```python
from build123d import *

# Parameters (mm, degrees)
EXTRUDE_1182_DEPTH                  = 20
SKETCH_1261_R                       = 9.7
SKETCH_1261_R_2                     = 8
EXTRUDE_1314_DEPTH                  = 25
EXTRUDE_1314_DIRECTION_2_REACH      = 36.873
EXTRUDE_1314_DIRECTION_2_END_RADIUS = 57.25
CUT_EXTRUDE_1_DEPTH                 = 54.783006673
CUT_EXTRUDE_1_DEPTH_BACK            = 54.783006673


with BuildPart() as part:
    # Sketch 176 → Extrude 1182 (new, symmetric)
    with BuildSketch(Plane.XY):
        with BuildLine():
            ThreePointArc((-7.173913043, 24.16738193), (-14.079724741, 13.582112358), (-16.5, 1.177257067))
            ThreePointArc((-16.5, 1.177257067), (0, -1.2), (16.5, 1.177257067))
            ThreePointArc((16.5, 1.177257067), (14.079724741, 13.582112358), (7.173913043, 24.16738193))
            ThreePointArc((7.173913043, 24.16738193), (0, 27.200677426), (-7.173913043, 24.16738193))
        make_face()
        with BuildLine():
            ThreePointArc((-0.89349881, 14.363604773), (-3.663033007, 7.517669831), (-4.022846329, 0.141513701))
            ThreePointArc((-4.022846329, 0.141513701), (-9.556707772, 0.803283208), (-15, 2))
            ThreePointArc((-15, 2), (-13.262165522, 12.062305899), (-8.25, 20.95883699))
            ThreePointArc((-8.25, 20.95883699), (-4.170568058, 18.108709455), (-0.89349881, 14.363604773))
        make_face(mode=Mode.SUBTRACT)
        with BuildLine():
            ThreePointArc((-2.5, 0.0546112), (-2.301572456, 6.695550977), (0, 12.928064021))
            ThreePointArc((0, 12.928064021), (2.301572456, 6.695550977), (2.5, 0.0546112))
            ThreePointArc((2.5, 0.0546112), (0, 0), (-2.5, 0.0546112))
        make_face(mode=Mode.SUBTRACT)
        with BuildLine():
            ThreePointArc((4.022846329, 0.141513701), (3.663033007, 7.517669831), (0.89349881, 14.363604773))
            ThreePointArc((0.89349881, 14.363604773), (4.170568058, 18.108709455), (8.25, 20.95883699))
            ThreePointArc((8.25, 20.95883699), (13.262165522, 12.062305899), (15, 2))
            ThreePointArc((15, 2), (9.556707772, 0.803283208), (4.022846329, 0.141513701))
        make_face(mode=Mode.SUBTRACT)
        with BuildLine():
            ThreePointArc((7.245751005, 22.120715085), (3.267177029, 19.312833939), (0, 15.701905849))
            ThreePointArc((0, 15.701905849), (-3.267177029, 19.312833939), (-7.245751005, 22.120715085))
            ThreePointArc((-7.245751005, 22.120715085), (0, 25.228756555), (7.245751005, 22.120715085))
        make_face(mode=Mode.SUBTRACT)
    extrude(amount=EXTRUDE_1182_DEPTH, both=True)

    # Sketch 1261 → Extrude 1314 (add)
    with BuildSketch(Plane(origin=(0, 22.120715085, 0), x_dir=(-1, 0, 0), z_dir=(0, -1, 0))):
        with Locations(Location((0, 0, 0), (0, 0, 222.304463408))):
            Circle(SKETCH_1261_R)
        with Locations(Location((0, 0, 0), (0, 0, 206.267303198))):
            Circle(SKETCH_1261_R_2, mode=Mode.SUBTRACT)
    extrude(amount=-EXTRUDE_1314_DEPTH)

    # Extrude 1314 direction 2: up to this cylinder (the profile starts inside it)
    extrude_1314_direction_2_end = Plane(origin=(0, 57.25, -6.344118), z_dir=(0, 0, -1)) * Cylinder(EXTRUDE_1314_DIRECTION_2_END_RADIUS, 189.246, mode=Mode.PRIVATE)
    # Sketch 1261 → Extrude 1314 direction 2 (add, up to the surface)
    with BuildSketch(Plane(origin=(0, 22.120715085, 0), x_dir=(-1, 0, 0), z_dir=(0, -1, 0)), mode=Mode.PRIVATE) as extrude_1314_direction_2_sk1:
        with Locations(Location((0, 0, 0), (0, 0, 222.304463408))):
            Circle(SKETCH_1261_R)
        with Locations(Location((0, 0, 0), (0, 0, 206.267303198))):
            Circle(SKETCH_1261_R_2, mode=Mode.SUBTRACT)
    extrude_1314_direction_2_tool1 = extrude(extrude_1314_direction_2_sk1.sketch, amount=EXTRUDE_1314_DIRECTION_2_REACH, mode=Mode.PRIVATE) & extrude_1314_direction_2_end
    add(extrude_1314_direction_2_tool1.solids().sort_by_distance((-6.971004, 22.120715, -6.344118))[0])

    # Sketch 1375 → 切除-拉伸1 (cut, two sides: drawn at the far end of the back side and taken through both)
    with BuildSketch(Plane.XY.offset(-CUT_EXTRUDE_1_DEPTH_BACK)):
        with BuildLine():
            ThreePointArc((4.022846329, 0.141513701), (9.556707772, 0.803283208), (15, 2))
            ThreePointArc((15, 2), (13.262165522, 12.062305899), (8.25, 20.95883699))
            ThreePointArc((8.25, 20.95883699), (4.170568058, 18.108709455), (0.89349881, 14.363604773))
            ThreePointArc((0.89349881, 14.363604773), (3.663033007, 7.517669831), (4.022846329, 0.141513701))
        make_face()
        with BuildLine():
            ThreePointArc((-8.25, 20.95883699), (-13.262165522, 12.062305899), (-15, 2))
            ThreePointArc((-15, 2), (-9.556707772, 0.803283208), (-4.022846329, 0.141513701))
            ThreePointArc((-4.022846329, 0.141513701), (-3.663033007, 7.517669831), (-0.89349881, 14.363604773))
            ThreePointArc((-0.89349881, 14.363604773), (-4.170568058, 18.108709455), (-8.25, 20.95883699))
        make_face()
        with BuildLine():
            ThreePointArc((-2.5, 0.0546112), (0, 0), (2.5, 0.0546112))
            ThreePointArc((2.5, 0.0546112), (2.301572456, 6.695550977), (0, 12.928064021))
            ThreePointArc((0, 12.928064021), (-2.301572456, 6.695550977), (-2.5, 0.0546112))
        make_face()
        with BuildLine():
            ThreePointArc((7.245751005, 22.120715085), (3.267177029, 19.312833939), (0, 15.701905849))
            ThreePointArc((0, 15.701905849), (-3.267177029, 19.312833939), (-7.245751005, 22.120715085))
            ThreePointArc((-7.245751005, 22.120715085), (0, 25.228756555), (7.245751005, 22.120715085))
        make_face()
    extrude(amount=CUT_EXTRUDE_1_DEPTH + CUT_EXTRUDE_1_DEPTH_BACK, mode=Mode.SUBTRACT)


solid = part.part
```
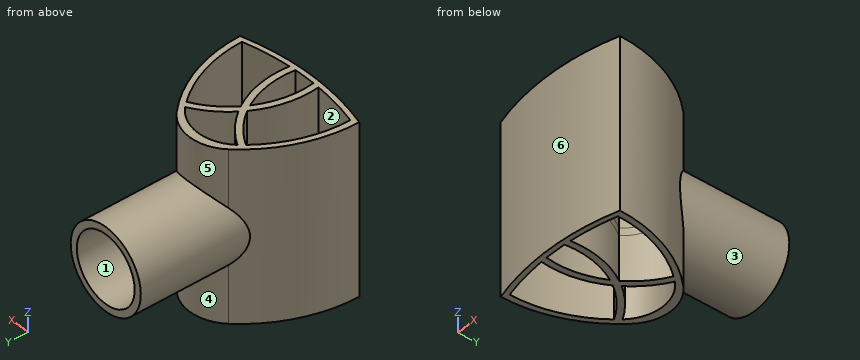
The listing builds one solid part. Answer for the finished solid, in the listing's coordinates (mm). Face numbers are marked on the shaded views. A direction names the side the tool comes from. Give positions to 0.01 mm unless a question says otherwise; leave off trailing zeros. Order: outer loops, then holes, each group sorted by start corner. A loop starts at its lowest first (then second) coordinate and runs counter-clockwise, first axis right, second up. Notation, with made-up numbers: (-27.5, 55) -> (-7.5, 55) arc R22 cw to (-7.5, 88) -> close; hole circle Ø3 at (76, 69.5). An arc over 180 degrees is marked (long way). One line per item, written item: value.
1) Flat-ended cylindrical pins translate along their axes: P1, Ø12, axis at x = 9.5, z = 1, coming from the -Y side; P2, Ø8, axis at x = 12, y = 34.5, coming from the -Z side; P3, Ø2, axis at x = -13, y = 11, coming from the +Z side; P4, Ø8, axis at y = 39, z = 2, coming from the +X side. Find the tip coordinate at first contact, or state that the pin passes through.
Reported:
P1: stops at y = -1.1
P2: stops at z = -5.49
P3: stops at z = 20
P4: stops at x = 9.7
2) Find section B-B, the plane y = 7.5. Determine the outline of the cut face in (x, z).
Reported:
outline: (-15.89, -20) -> (-14.49, -20) -> (-14.49, 20) -> (-15.89, 20) -> close; (-3.67, -20) -> (-2.13, -20) -> (-2.13, 20) -> (-3.67, 20) -> close; (2.13, -20) -> (3.67, -20) -> (3.67, 20) -> (2.13, 20) -> close; (14.49, -20) -> (15.89, -20) -> (15.89, 20) -> (14.49, 20) -> close
3) Find section A-A, the plane z = -13.5. Determine the outline of the cut face in (x, y).
Reported:
outline: (-16.5, 1.18) arc R58.45 ccw to (16.5, 1.18) arc R33 ccw to (7.17, 24.17) arc R10 ccw to (-7.17, 24.17) arc R33 ccw to start; hole (-15, 2) arc R57.25 ccw to (-4.02, 0.14) arc R22.1 cw to (-0.89, 14.36) arc R20.6 ccw to (-8.25, 20.96) arc R30 ccw to start; hole (-7.25, 22.12) arc R22.1 cw to (0, 15.7) arc R22.1 cw to (7.25, 22.12) arc R10 ccw to start; hole (-2.5, 0.05) arc R57.25 ccw to (2.5, 0.05) arc R20.6 ccw to (0, 12.93) arc R20.6 ccw to start; hole (0.89, 14.36) arc R22.1 cw to (4.02, 0.14) arc R57.25 ccw to (15, 2) arc R30 ccw to (8.25, 20.96) arc R20.6 ccw to start
4) Find section C-C, the plane x = -14. Determine the outline of the cut face in (y, z).
Reported:
outline: (0.5, -20) -> (1.74, -20) -> (1.74, 20) -> (0.5, 20) -> close; (9.68, -20) -> (13.78, -20) -> (13.78, 20) -> (9.68, 20) -> close
5) Determine the mould class of the marked faces 1, 2 and 3 for opening direction Z: pulls with the +Z half, pulls with the -Z half, needs draft (parallel to the pull), parting line crosses it, or undercut.
Reported:
face 1: undercut
face 2: needs draft
face 3: parting line crosses it
6) A tool of negligible diameter and unlimited length cuts with its end or side. For the marked faces 4, 5 and 6, from which of +Z, -Z, +X, -X, +Y, -Y can it reach the whole face along a straight path? Write none if from no direction.
Reported:
face 4: -Z, +Y
face 5: +Z, +Y
face 6: +Z, -Z, -Y
7) Find section D-D, the plane y = 13.5. Determine the outline of the cut face in (x, z), plus the area to 3 significant figures.
Reported:
outline: (-14.11, -20) -> (-12.71, -20) -> (-12.71, 20) -> (-14.11, 20) -> close; (-1.4, -20) -> (1.4, -20) -> (1.4, 20) -> (-1.4, 20) -> close; (12.71, -20) -> (14.11, -20) -> (14.11, 20) -> (12.71, 20) -> close
area: 224 mm^2
8) Find the intervals of material crossed by line 1 (X direction, y = 29, z = 0); line 2 (X direction, y = 7.5, z = -2.5), in increasing order.
Reported:
line 1: x = -9.7 to -8, 8 to 9.7
line 2: x = -15.89 to -14.49, -3.67 to -2.13, 2.13 to 3.67, 14.49 to 15.89
